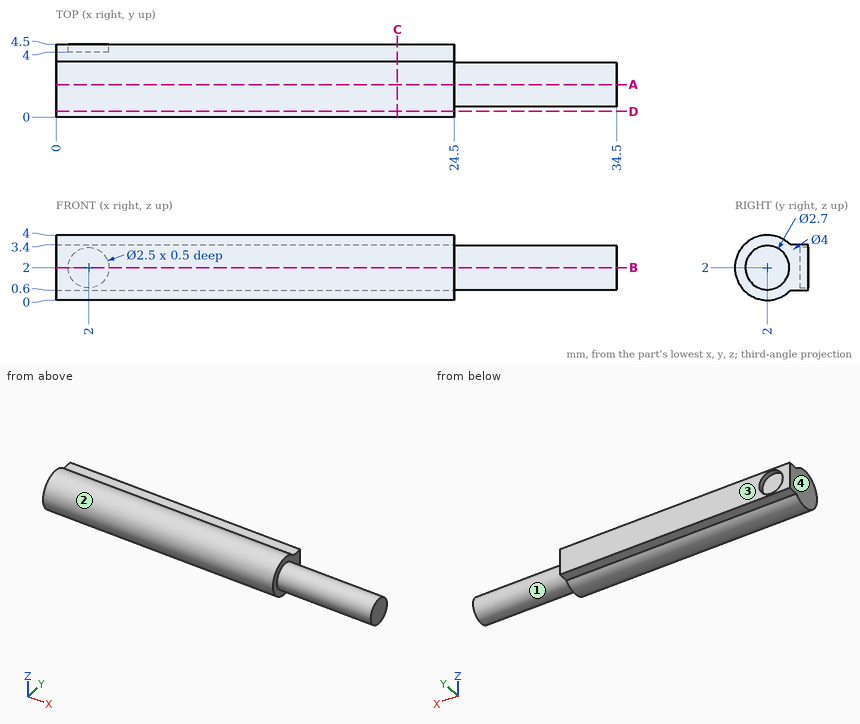
Design review of the part shown in the three views and the two pictorial views. Dimensions are in mm from the part's minimum x, y and z. A direction names the side the tool comes from. Coordinates: 2 decimals unless noted, no trailing zeros. Loops run counter-clockwise (first coordinate to the right, second up) from the corner with the lowest first, then second, coordinate; pieces in that order, holes last. Notation, with made-up numbers: M 24,12 L 70,12 A18 ccw 70,22 Z; hole C -32.5,45.25 d11. An arc over 180 degrees is marked long. Put each result on its own line as item: value. Start each with the question number.
Q1. Add section C-C (x = 21). Write out the cut boundary in (y, z).
Q2. Add section D-D (y = 0.35). Write out the cut boundary in (x, z).
Q3. Clearance check with flat-ended pins moving along their axes: pin 1 (2 mm diameter, centred on x = 30.5, y = 4, fed in from -Z); pin 2 (1.2 mm diameter, centred on x = 9.5, y = 4, fed in from -Z); pin 3 (0.5 mm diameter, centred on x = 14, y = 4, fed in from +Z). State where each tip first meets the part, or that it passes through.
Q4. The part is to be moulded in two halves that separate along X. For the marked faces 3 and 4, say which applies: +X half, -X half, draft (parallel to the pull), parting line (faces both ways), or undercut.
Q5. Add section B-B (z = 2). Write out the cut boundary in (x, y).
Q6. Wall thickness on line 1 (X direction, y = 4.15, z = 2); line 2 (X direction, y = 1.05, z = 0.35); line 3 (Z direction, x = 16, y = 3.95): over which ranges is each line inside the solid? List them lowest first.
Q7. For the marked faces 1 and 2, list the 3-axis set-ups (+Z, -Z, +X, -X, +Y, -Y) from which the entire face can be reached by the end or side of a thin tool; tool diameter is ignored.
Q8. Add section A-A (y = 2). Write out the cut boundary in (x, z), and give its area (3 significant figures).
Answers:
1. outline: M 3.43,0.6 L 4.5,0.6 L 4.5,3.4 L 3.43,3.4 A2 ccw long Z
2. outline: M 0,0.87 L 24.5,0.87 L 24.5,3.13 L 0,3.13 Z
3. pin 1: stops at z = 1.09
3. pin 2: stops at z = 0.57
3. pin 3: stops at z = 3.4
4. face 3: draft
4. face 4: -X half
5. outline: M 0,0 L 24.5,0 L 24.5,0.65 L 34.5,0.65 L 34.5,3.35 L 24.5,3.35 L 24.5,4.5 L 3.25,4.5 L 3.25,4 L 0.75,4 L 0.75,4.5 L 0,4.5 Z
6. line 1: x = 0 to 0.75, 3.25 to 24.5
6. line 2: x = 0 to 24.5
6. line 3: z = 0.6 to 3.4
7. face 1: +X
7. face 2: +X, -X
8. outline: M 0,0 L 24.5,0 L 24.5,0.65 L 34.5,0.65 L 34.5,3.35 L 24.5,3.35 L 24.5,4 L 0,4 Z
8. area: 125 mm^2
